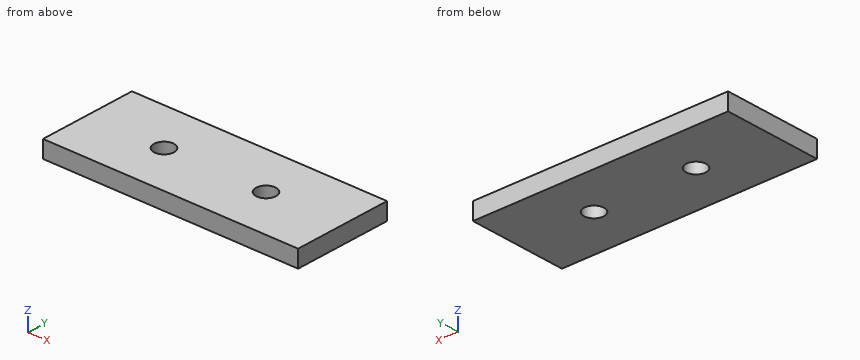
```python
from build123d import *

# Parameters (mm, degrees)
SKETCH1_W            = 90
SKETCH1_H            = 35
BOSS_EXTRUDE1_DEPTH  = 6
M6_CLEARANCE_HOLE1_D = 7


with BuildPart() as part:
    # Sketch1 → Boss-Extrude1 (new body)
    with BuildSketch(Plane.XY):
        with Locations((45, 17.5)):
            Rectangle(SKETCH1_W, SKETCH1_H)
    extrude(amount=BOSS_EXTRUDE1_DEPTH)

    # M6 Clearance Hole1 (through all)
    with Locations(Plane.XY.offset(6)):
        with Locations((27, 17.5), (63, 17.5)):
            Hole(M6_CLEARANCE_HOLE1_D / 2)


solid = part.part
```
For this review, take the finished solid that the model builds, in its own axes (mm). Round coordinates to 2 decimals unless told otherwise and drop trailing zeros. Write each loop counter-clockwise with the first axis right and the second up, starting at its lowest first coordinate (ties: lowest second). Pieces come first, ordered by that corner, then holes. Notation, with made-up numbers: (60.25, -30.75) - (70.25, -30.75) arc R12 ccw to (70.25, -10.75) - close; hole circle Ø11 at (76.5, 23.5). An arc over 180 degrees is marked (long way). Answer as a JSON object with one key per item and string values.
1. We need section C-C on z = 3.1. Give the boundary of the cut face in (x, y), then the cut area to 3 significant figures.
Response values:
{"outline": "(0, 0) - (90, 0) - (90, 35) - (0, 35) - close; hole circle Ø7 at (27, 17.5); hole circle Ø7 at (63, 17.5)", "area": "3,070 mm2"}
2. To check wall thickness, follow line 1 along Y through (x, z) = (27, 3.85); line 2 along X through (y, z) = (19.5, 5.65); line 3 along X through (y, z) = (15, 5.5). State the ranges of each line that lie inside material, in increasing order.
Response values:
{"line 1": "y = 0 to 14, 21 to 35", "line 2": "x = 0 to 24.13, 29.87 to 60.13, 65.87 to 90", "line 3": "x = 0 to 24.55, 29.45 to 60.55, 65.45 to 90"}
3. For pin 1 Ø5.5 at (x, y) = (27, 17.5) entering from +Z, flat-tipped, find the tip position at first contact; note if it passes through.
Response values:
{"pin 1": "passes through"}
4. We need section A-A on y = 17.5. Give the boundary of the cut face in (x, z).
Response values:
{"outline": "(0, 0) - (23.5, 0) - (23.5, 6) - (0, 6) - close; (30.5, 0) - (59.5, 0) - (59.5, 6) - (30.5, 6) - close; (66.5, 0) - (90, 0) - (90, 6) - (66.5, 6) - close"}
5. We need section B-B on x = 27. Give the boundary of the cut face in (y, z).
Response values:
{"outline": "(0, 0) - (14, 0) - (14, 6) - (0, 6) - close; (21, 0) - (35, 0) - (35, 6) - (21, 6) - close"}
